```python
from build123d import *

# Parameters (mm, degrees)
BOSS_EXTRUDE1_DEPTH = 38
BOSS_EXTRUDE2_DEPTH = 2
BOSS_EXTRUDE3_DEPTH = 2
SKETCH4_R           = 4.25
CUT_EXTRUDE1_DEPTH  = 66.337584896
CUT_EXTRUDE2_DEPTH  = 69.14690015


with BuildPart() as part:
    # Sketch1 → Boss-Extrude1 (new body)
    with BuildSketch(Plane.XY):
        Polygon((0, 0), (40, 0), (40, 5), (5, 5), (5, 40), (0, 40), align=None)
    extrude(amount=BOSS_EXTRUDE1_DEPTH)

    # Sketch2 → Boss-Extrude2 (add)
    with BuildSketch(Plane.XY.offset(38)):
        Polygon((7, 40), (7, 38), (38, 7), (40, 7), (40, 5), (5, 5), (5, 40), align=None)
    extrude(amount=-BOSS_EXTRUDE2_DEPTH)

    # Sketch3 → Boss-Extrude3 (add)
    with BuildSketch(Plane(origin=(0, 0, 0), x_dir=(-1, 0, 0), z_dir=(0, 0, -1))):
        Polygon((-38, 7), (-7, 38), (-7, 40), (-5, 40), (-5, 5), (-40, 5), (-40, 7), align=None)
    extrude(amount=-BOSS_EXTRUDE3_DEPTH)

    # Sketch4 → Cut-Extrude1 (cut, through all)
    with BuildSketch(Plane(origin=(0, 5, 0), x_dir=(1, 0, 0), z_dir=(0, 1, 0))):
        with Locations(Location((22.5, -19, 0), (0, 0, 270))):
            Circle(SKETCH4_R)
    extrude(amount=-CUT_EXTRUDE1_DEPTH, mode=Mode.SUBTRACT)

    # Sketch5 → Cut-Extrude2 (cut, through all)
    with BuildSketch(Plane.ZY):
        with BuildLine():
            Line((14.75, 22.5), (14.75, 18.25))
            ThreePointArc((14.75, 18.25), (19, 14), (23.25, 18.25))
            Line((23.25, 18.25), (23.25, 26.75))
            ThreePointArc((23.25, 26.75), (19, 31), (14.75, 26.75))
            Line((14.75, 26.75), (14.75, 22.5))
        make_face()
    extrude(amount=-CUT_EXTRUDE2_DEPTH, mode=Mode.SUBTRACT)


solid = part.part
```
Geometry check sheet. Reference: the model listing, model coordinates, mm. A direction names the side the tool comes from. Give positions to 0.01 mm unless a question says otherwise; leave off trailing zeros. Order: outer loops, then holes, each group sorted by start corner. A loop starts at its lowest first (then second) coordinate and runs counter-clockwise, first axis right, second up.
1. Gauge pin test, flat ends, axial feed: pin 1 Ø10 at (x, z) = (23, 22) entering from +Y; pin 2 Ø2 at (x, z) = (39.5, 1) entering from +Y; pin 3 Ø1 at (y, z) = (39.5, 1.5) entering from +X. Record the tip position at first contact, or that the pin passes through.
2. Access from +Z, -Z, +X, -X, +Y, -Y to the whole of each face (thin tool, end or side, straight path). Record for faces 4 (the face through (2, 23, 14.75)), 5 (the face through (39, 7, 37)), 6 (the face through (15, 15, 36)).
3. Thickness scan on L1, parallel to X at y = 2.45, z = 19; L2, parallel to Z at x = 7, y = 8; L3, parallel to Z at x = 22, y = 1. Record the ranges inside material, lowest first.
4. Release check for a two-part mould opening along Y. For faces 1 (the face through (39, 7, 1)), 2 (the face through (19.91, 2.54, 15.63)), 3 (the face through (2, 14, 19)) record: pulls with the +Y half, pulls with the -Y half, needs draft (parallel to the pull), parting line crosses it, or undercut.
5. Section check A-A, the plane z = 19. Enter the section's corners in (x, y), and give its area (4 significant figures).
6. Section check C-C, the plane x = 27.5. Enter the section's corners in (y, z).
7. Section check B-B, the plane y = 26. Enter the section's corners in (x, z).
8. Section check D-D, the plane x = 22.5. Enter the section's corners in (y, z).
Values follow:
1. pin 1: stops at y = 5
1. pin 2: stops at y = 7
1. pin 3: stops at x = 7
2. face 4: +X, -X
2. face 5: +Z, -Z, +X, +Y
2. face 6: +X, +Y
3. L1: x = 0 to 18.25, 26.75 to 40
3. L2: z = 0 to 2, 36 to 38
3. L3: z = 0 to 14.78, 23.22 to 38
4. face 1: pulls with the +Y half
4. face 2: needs draft
4. face 3: undercut
5. outline: (0, 0) - (18.25, 0) - (18.25, 5) - (5, 5) - (5, 14) - (0, 14) - close; (0, 31) - (5, 31) - (5, 40) - (0, 40) - close; (26.75, 0) - (40, 0) - (40, 5) - (26.75, 5) - close
5. area: 247.5 mm2
6. outline: (0, 0) - (17.5, 0) - (17.5, 2) - (5, 2) - (5, 36) - (17.5, 36) - (17.5, 38) - (0, 38) - close
7. outline: (0, 0) - (19, 0) - (19, 2) - (5, 2) - (5, 14.75) - (0, 14.75) - close; (0, 23.25) - (5, 23.25) - (5, 36) - (19, 36) - (19, 38) - (0, 38) - close
8. outline: (0, 0) - (22.5, 0) - (22.5, 2) - (5, 2) - (5, 14.75) - (0, 14.75) - close; (0, 23.25) - (5, 23.25) - (5, 36) - (22.5, 36) - (22.5, 38) - (0, 38) - close
